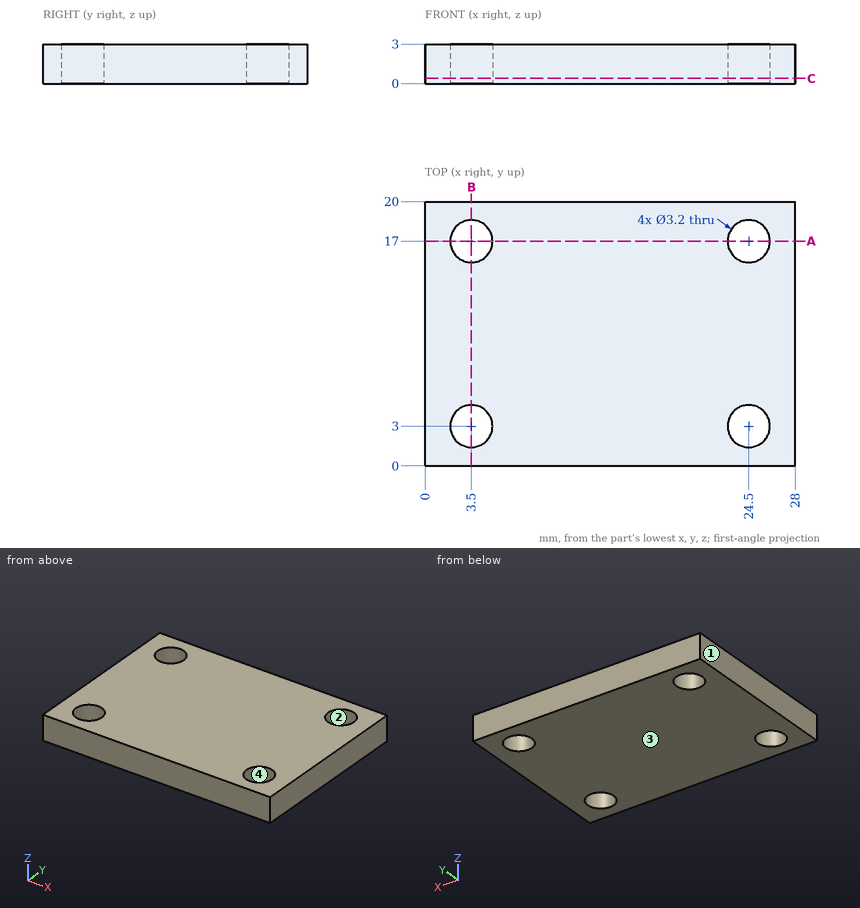
Job drawing, mm, ordinate dimensions from the low corner. One solid piece. Coordinates: 2 decimals unless noted, no trailing zeros. Order: outer loops, then holes, each group sorted by start corner. A loop starts at its lowest first (then second) coordinate and runs counter-clockwise, first axis right, second up. Notation, with made-up numbers: (79, -2) - (105, -2) arc R15 ccw to (105, 10) - close; hole circle Ø1 at (16.5, 23). An arc over 180 degrees is marked (long way). Write each question's results on one line, items separated by ' | '. Start each with the question number.
Item 1: Band-saw the part on C-C on z = 0.4. Write the cut outline in (x, y).
Item 2: Wall check: probe 1 along Y at (x, z) = (24.5, 1.9); probe 2 along X at (y, z) = (2, 2.85); probe 3 along X at (y, z) = (16.25, 2.75). Give the ranges that are in metal, low to high. Write a range as [from, to].
Item 3: Band-saw the part on B-B on x = 3.5. Write the cut outline in (y, z).
Item 4: Mould opens along X. For the marked faces 1, 2, 3 and 4 say: released by +X, released by -X, zero draft, split by the parting line, or undercut.
Item 5: Band-saw the part on A-A on y = 17. Write the cut outline in (x, z), and give its area (3 significant figures).
Numbers:
1) outline: (0, 0) - (28, 0) - (28, 20) - (0, 20) - close; hole circle Ø3.2 at (3.5, 3); hole circle Ø3.2 at (3.5, 17); hole circle Ø3.2 at (24.5, 3); hole circle Ø3.2 at (24.5, 17)
2) probe 1: [0, 1.4], [4.6, 15.4], [18.6, 20] | probe 2: [0, 2.25], [4.75, 23.25], [25.75, 28] | probe 3: [0, 2.09], [4.91, 23.09], [25.91, 28]
3) outline: (0, 0) - (1.4, 0) - (1.4, 3) - (0, 3) - close; (4.6, 0) - (15.4, 0) - (15.4, 3) - (4.6, 3) - close; (18.6, 0) - (20, 0) - (20, 3) - (18.6, 3) - close
4) face 1: released by -X | face 2: undercut | face 3: zero draft | face 4: undercut
5) outline: (0, 0) - (1.9, 0) - (1.9, 3) - (0, 3) - close; (5.1, 0) - (22.9, 0) - (22.9, 3) - (5.1, 3) - close; (26.1, 0) - (28, 0) - (28, 3) - (26.1, 3) - close | area: 64.8 mm^2
